```python
from build123d import *

# Parameters (mm, degrees)
BOSS_EXTRUDE1_DEPTH                                 = 7
SKETCH2_R                                           = 1
CUT_EXTRUDE1_DEPTH                                  = 77.798437484
SKETCH3_W                                           = 5
SKETCH3_H                                           = 10
CUT_EXTRUDE2_DEPTH                                  = 71.563800918
SKETCH4_R                                           = 2
CUT_EXTRUDE3_DEPTH                                  = 75.652528423
M3_TAPPED_HOLE1_REACH                               = 72.564
M3_TAPPED_HOLE1_BORE_R                              = 1.25
FILLET1_R                                           = 4
CHAMFER1_SIZE                                       = 1
SKETCH8_R                                           = 4
CUT_EXTRUDE4_DEPTH                                  = 2
FILLET2_R                                           = 2
M2_TAPPED_HOLE1_D                                   = 1.6
M2_TAPPED_HOLE1_DEPTH                               = 5.2
M2_TAPPED_HOLE1_TIP                                 = 0.480688495
CBORE_FOR_M3_HEX_SOCKET_HEAD_CAP_SCREW1_D           = 3.4
CBORE_FOR_M3_HEX_SOCKET_HEAD_CAP_SCREW1_CBORE_D     = 6.5
CBORE_FOR_M3_HEX_SOCKET_HEAD_CAP_SCREW1_CBORE_DEPTH = 3.4


with BuildPart() as part:
    # Sketch1 → Boss-Extrude1 (new body)
    with BuildSketch(Plane.XY):
        Polygon((17.5, 0), (-17.5, 0), (-17.5, 68), (-12, 68), (-12, 36), (12, 36), (12, 68), (17.5, 68), align=None)
    extrude(amount=BOSS_EXTRUDE1_DEPTH)

    # Sketch2 → Cut-Extrude1 (cut, through all)
    with BuildSketch(Plane(origin=(17.5, 0, 0), x_dir=(0, 0, -1), z_dir=(1, 0, 0))):
        with Locations((-2, 65.5)):
            Circle(SKETCH2_R)
    extrude(amount=-CUT_EXTRUDE1_DEPTH, mode=Mode.SUBTRACT)

    # Sketch3 → Cut-Extrude2 (cut, through all)
    with BuildSketch(Plane.XY.offset(7)):
        with Locations((-15, 5)):
            Rectangle(SKETCH3_W, SKETCH3_H)
        with Locations((15, 5)):
            Rectangle(SKETCH3_W, SKETCH3_H)
    extrude(amount=-CUT_EXTRUDE2_DEPTH, mode=Mode.SUBTRACT)

    # Sketch4 → Cut-Extrude3 (cut, through all)
    with BuildSketch(Plane(origin=(12.5, 0, 0), x_dir=(0, 0, -1), z_dir=(1, 0, 0))):
        with Locations((-3.5, 4)):
            Circle(SKETCH4_R)
    extrude(amount=-CUT_EXTRUDE3_DEPTH, mode=Mode.SUBTRACT)

    # M3 Tapped Hole1 bore → M3 Tapped Hole1 (cut, up to next)
    with BuildSketch(Plane.XZ, mode=Mode.PRIVATE) as m3_tapped_hole1_sk1:
        with Locations((7.5, 3.5)):
            Circle(M3_TAPPED_HOLE1_BORE_R)
    m3_tapped_hole1_tool1 = extrude(m3_tapped_hole1_sk1.sketch, amount=-M3_TAPPED_HOLE1_REACH, mode=Mode.PRIVATE) & part.part
    # M3 Tapped Hole1 bore → M3 Tapped Hole1 (cut, up to next)
    with BuildSketch(Plane.XZ, mode=Mode.PRIVATE) as m3_tapped_hole1_sk2:
        with Locations((-7.5, 3.5)):
            Circle(M3_TAPPED_HOLE1_BORE_R)
    m3_tapped_hole1_tool2 = extrude(m3_tapped_hole1_sk2.sketch, amount=-M3_TAPPED_HOLE1_REACH, mode=Mode.PRIVATE) & part.part
    add(m3_tapped_hole1_tool1.solids().sort_by_distance((7.5, 0, 3.5))[0], mode=Mode.SUBTRACT)
    add(m3_tapped_hole1_tool2.solids().sort_by_distance((-7.5, 0, 3.5))[0], mode=Mode.SUBTRACT)

    # Fillet1
    fillet1_edges = [part.edges().sort_by_distance(p)[0] for p in [
        (-12, 36, 3.5),
        (12, 36, 3.5),
    ]]
    fillet(fillet1_edges, radius=FILLET1_R)

    # Chamfer1
    chamfer1_edges = [part.edges().sort_by_distance(p)[0] for p in [
        (14.75, 68, 7),
        (-14.75, 68, 7),
        (-17.5, 10, 3.5),
        (17.5, 10, 3.5),
    ]]
    chamfer(chamfer1_edges, length=CHAMFER1_SIZE)

    # Sketch8 → Cut-Extrude4 (cut)
    with BuildSketch(Plane.XY.offset(7)):
        with Locations((0, 18)):
            Circle(SKETCH8_R)
    extrude(amount=-CUT_EXTRUDE4_DEPTH, mode=Mode.SUBTRACT)

    # Fillet2
    fillet2_edges = [part.edges().sort_by_distance(p)[0] for p in [
        (-14.75, 68, 0),
        (14.75, 68, 0),
    ]]
    fillet(fillet2_edges, radius=FILLET2_R)

    # M2 Tapped Hole1
    with Locations(Plane.XY.offset(7)):
        with Locations((-14.75, 65.5), (14.75, 65.5)):
            Hole(M2_TAPPED_HOLE1_D / 2, depth=M2_TAPPED_HOLE1_DEPTH)
            with Locations((0, 0, -(M2_TAPPED_HOLE1_DEPTH + M2_TAPPED_HOLE1_TIP / 2))):  # 118° drill point
                Cone(0, M2_TAPPED_HOLE1_D / 2, M2_TAPPED_HOLE1_TIP, mode=Mode.SUBTRACT)

    # CBORE for M3 Hex Socket Head Cap Screw1 (through all)
    with Locations(Plane(origin=(0, 0, 0), x_dir=(-1, 0, 0), z_dir=(0, 0, -1))):
        with Locations((0, 18)):
            CounterBoreHole(CBORE_FOR_M3_HEX_SOCKET_HEAD_CAP_SCREW1_D / 2, CBORE_FOR_M3_HEX_SOCKET_HEAD_CAP_SCREW1_CBORE_D / 2, CBORE_FOR_M3_HEX_SOCKET_HEAD_CAP_SCREW1_CBORE_DEPTH)


solid = part.part
```
Input: part model. Units: mm. Frame: model coordinates. A direction names the side the tool comes from. Round coordinates to 2 decimals unless told otherwise and drop trailing zeros. Loops run counter-clockwise (first coordinate to the right, second up) from the corner with the lowest first, then second, coordinate; pieces in that order, holes last. Notation, with made-up numbers: M 30.25,69.5 L 77.25,69.5 A13 cw 77.25,80.5 Z; hole C -23,8 d8. An arc over 180 degrees is marked long. Answer in a Markdown table with one row per item. Add a question column.
1. Contact query for flat-ended pins moving along their axis: pin 1 (5 mm diameter, centred on x = -9.5, y = 35, fed in from -Z); pin 2 (3.5 mm diameter, centred on y = 6, z = 4, fed in from +X); pin 3 (4 mm diameter, centred on x = -1, z = 6, fed in from +Y); pin 4 (3 mm diameter, centred on x = -7.5, z = 3.5, fed in from +Y). Output: stop coordinate, or through.
2. Mould query, pull axis X, two halves, no side actions, for faces 1 (the face through (-12, 54, 3)), 2 (the face through (-14.712, 65.117, 1.076)), 3 (the face through (17.5, 40, 3)). Classes: released by +X, released by -X, zero draft, split by the parting line, or undercut.
3. Section C-C (x = -14.75). Output: boundary loops of the cut face in (y, z), and give its area (3 significant figures).
4. Section D-D (y = 44). Output: boundary loops of the cut face in (x, z).
5. Set-up query: faces 4 (the face through (12.5, 6, 4.3)), 5 (the face through (-15.489, 65.194, 4.769)), 6 (the face through (-6.31, 1.2, 3.88)). Return all of +Z, -Z, +X, -X, +Y, -Y with unobstructed straight access to the full face (end or side cutting, diameter ignored); none if empty.
6. Ray query, probe 1 along X at (y, z) = (1.15, 3.5); probe 2 along X at (y, z) = (51, 0.75); probe 3 along Y at (x, z) = (15.8, 2). Return the intervals inside material, ascending.
7. Section B-B (y = 4). Output: boundary loops of the cut face in (x, z), and give its area (3 significant figures).
8. Section A-A (x = 0). Output: boundary loops of the cut face in (y, z), and give its area (3 significant figures).
Values follow:
| question | item | result |
|---|---|---|
| 1 | pin 1 | z = 0 |
| 1 | pin 2 | x = 12.5 |
| 1 | pin 3 | y = 36 |
| 1 | pin 4 | y = 36.13 |
| 2 | face 1 | undercut |
| 2 | face 2 | zero draft |
| 2 | face 3 | released by +X |
| 3 | outline | M 10,0 L 66,0 A2 ccw 68,2 L 68,6 L 67,7 L 66.3,7 L 66.3,2.6 A1 cw long 64.7,2.6 L 64.7,7 L 10,7 Z |
| 3 | area | 395 mm^2 |
| 4 | outline | M -17.5,0 L -12,0 L -12,7 L -17.5,7 Z; M 12,0 L 17.5,0 L 17.5,7 L 12,7 Z |
| 5 | face 4 | +Z, -Z, +X, -Y |
| 5 | face 5 | +Z |
| 5 | face 6 | -Y |
| 6 | probe 1 | -12.5 to -8.75, -6.25 to 6.25, 8.75 to 12.5 |
| 6 | probe 2 | -17.5 to -12, 12 to 17.5 |
| 6 | probe 3 | 10 to 64.5, 66.5 to 68 |
| 7 | outline | M -12.5,0 L 12.5,0 L 12.5,1.5 L -12.5,1.5 Z; M -12.5,5.5 L 12.5,5.5 L 12.5,7 L -12.5,7 Z |
| 7 | area | 75.0 mm^2 |
| 8 | outline | M 0,0 L 14.75,0 L 14.75,3.4 L 16.3,3.4 L 16.3,5 L 14,5 L 14,7 L 0,7 Z; M 19.7,3.4 L 21.25,3.4 L 21.25,0 L 36,0 L 36,7 L 22,7 L 22,5 L 19.7,5 Z; hole C 4,3.5 d4 |
| 8 | area | 196 mm^2 |
